Can you work these out from the model? Positions are in its coordinate system, mm. A direction names the side the tool comes from. Coordinates: 2 decimals unless noted, no trailing zeros. Loops run counter-clockwise (first coordinate to the right, second up) from the corner with the lowest first, then second, coordinate; pieces in that order, holes last. Notation, with made-up numbers: (60.25, -27.5) -> (94.25, -27.5) arc R6 ccw to (94.25, -21.5) -> close; hole circle Ø2 at (-1, -5.75). An arc over 180 degrees is marked (long way). Put each result on its own line as item: value. Start each with the question number.
Item 1: We'd pull the mould along X, two halves only. Please class faces 5 (the cylindrical face through (13.1, 7.58, 2.96)), 6 (the flat face through (0, -16.5, -32)), 7 (the flat face through (-20, 0, 3)): pulls with the +X half, pulls with the -X half, needs draft (parallel to the pull), parting line crosses it, or undercut.
Item 2: If we section it at D-D on x = 6.5: Please give me the cut outline in (y, z).
Item 3: If we section it at B-B on y = 158.5: Please give me the cut outline in (x, z).
Item 4: Will these pins go through, and if not, where does the flat tip stop? P1, Ø8, axis at x = 11.5, z = -10, coming from the +Y side; P2, Ø4.5, axis at x = -15, y = 7.5, coming from the -Z side; P3, Ø3, axis at x = 4, z = 1.5, coming from the -Y side; P4, Ø8, axis at x = -10.5, y = 13, coming from the +Z side.
Item 5: If we section it at C-C on z = -39: Please give me the cut outline in (x, y), plus the area to 3 significant figures.
Item 6: For faces 1 (the flat face through (10, 64, -32)), 2 (the flat face through (16, 153, -10)), 3 (the flat face through (-10, 65, -32)), 4 (the flat face through (0, -12.5, 3)), which set-ups out of +Z, -Z, +X, -X, +Y, -Y let a thin tool reach every point of the face, with its end or its side?
Item 7: Please list where these lines run through material, in increasing order: L1, parallel to Y at x = -15, z = 3.4; L2, parallel to X at y = -7, z = 2; L3, parallel to Y at x = 1.5, z = -49. Write a range as from..to.
Item 8: If we section it at A-A on z = -12.5: Please give me the cut outline in (x, y), plus the area to 3 significant figures.
```python
from build123d import *

# Parameters (mm, degrees)
SKETCH1_R                = 1.9
BOSS_EXTRUDE1_DEPTH      = 6
SKETCH2_W                = 18
SKETCH2_H                = 13
BOSS_EXTRUDE2_DEPTH      = 32
BOSS_EXTRUDE3_DEPTH      = 10
BOSS_EXTRUDE3_DEPTH_BACK = 150
SKETCH4_W                = 20
SKETCH4_H                = 26
BOSS_EXTRUDE4_DEPTH      = 10
BOSS_EXTRUDE4_DEPTH_BACK = 35
SKETCH5_R                = 19
SKETCH5_R_2              = 15
FILLET1_R                = 0.8


with BuildPart() as part:
    # Sketch1 → Boss-Extrude1 (new body)
    with BuildSketch(Plane.XY):
        with BuildLine():
            Line((-16, 12.5), (16, 12.5))
            ThreePointArc((16, 12.5), (18.828427125, 11.328427125), (20, 8.5))
            Line((20, 8.5), (20, -8.5))
            ThreePointArc((20, -8.5), (18.828427125, -11.328427125), (16, -12.5))
            Line((16, -12.5), (-16, -12.5))
            ThreePointArc((-16, -12.5), (-18.828427125, -11.328427125), (-20, -8.5))
            Line((-20, -8.5), (-20, 8.5))
            ThreePointArc((-20, 8.5), (-18.828427125, 11.328427125), (-16, 12.5))
        make_face()
        with Locations((-15, 7.5)):
            Circle(SKETCH1_R, mode=Mode.SUBTRACT)
        with Locations((15, 7.5)):
            Circle(SKETCH1_R, mode=Mode.SUBTRACT)
        with Locations((15, -7.5)):
            Circle(SKETCH1_R, mode=Mode.SUBTRACT)
        with Locations((-15, -7.5)):
            Circle(SKETCH1_R, mode=Mode.SUBTRACT)
    extrude(amount=BOSS_EXTRUDE1_DEPTH)

    # Sketch2 → Boss-Extrude2 (add)
    with BuildSketch(Plane(origin=(0, 0, 0), x_dir=(-1, 0, 0), z_dir=(0, 0, -1))):
        Rectangle(SKETCH2_W, SKETCH2_H)
    extrude(amount=BOSS_EXTRUDE2_DEPTH)

    # Sketch4 → Boss-Extrude3 (add, two sides: drawn at the far end of the back side and taken through both)
    with BuildSketch(Plane(origin=(0, -6.5, 0), x_dir=(-1, 0, 0), z_dir=(0, -1, 0)).offset(-BOSS_EXTRUDE3_DEPTH_BACK)):
        with Locations((0, 32)):
            Rectangle(SKETCH4_W, SKETCH4_H)
    extrude(amount=BOSS_EXTRUDE3_DEPTH + BOSS_EXTRUDE3_DEPTH_BACK)

    # Sketch5 → Boss-Extrude4 (add, two sides: drawn at the far end of the back side and taken through both)
    with BuildSketch(Plane(origin=(0, 0, -45), x_dir=(-1, 0, 0), z_dir=(0, 0, -1)).offset(-BOSS_EXTRUDE4_DEPTH_BACK)):
        with Locations((-1.66190379, 158.5)):
            Circle(SKETCH5_R)
        with Locations((-1.66190379, 158.5)):
            Circle(SKETCH5_R_2, mode=Mode.SUBTRACT)
    extrude(amount=BOSS_EXTRUDE4_DEPTH + BOSS_EXTRUDE4_DEPTH_BACK)

    # Fillet1
    fillet1_edges = [part.edges().sort_by_distance(p)[0] for p in [
        (-9, -6.5, -9.5),
        (9, -6.5, -9.5),
        (9, 6.5, -9.5),
        (-9, 6.5, -9.5),
        (-10, 63.5, -19),
        (-10, 63.5, -45),
        (10, -16.5, -32),
        (0, -16.5, -19),
        (-10, -16.5, -32),
        (0, -16.5, -45),
        (10, 62.463663672, -45),
        (10, 62.463663672, -19),
    ]]
    fillet(fillet1_edges, radius=FILLET1_R)


solid = part.part
```
Solutions:
1. face 5: undercut
1. face 6: needs draft
1. face 7: pulls with the -X half
2. outline: (-16.5, -44.2) arc R0.8 ccw to (-15.7, -45) -> (140.13, -45) -> (140.13, -55) -> (144.3, -55) -> (144.3, -10) -> (140.13, -10) -> (140.13, -19) -> (6.5, -19) -> (6.5, 0) -> (12.5, 0) -> (12.5, 6) -> (-12.5, 6) -> (-12.5, 0) -> (-6.5, 0) -> (-6.5, -19) -> (-15.7, -19) arc R0.8 ccw to (-16.5, -19.8) -> close; (172.7, -55) -> (176.87, -55) -> (176.87, -10) -> (172.7, -10) -> close
3. outline: (-17.34, -55) -> (-13.34, -55) -> (-13.34, -10) -> (-17.34, -10) -> close; (16.66, -55) -> (20.66, -55) -> (20.66, -10) -> (16.66, -10) -> close
4. P1: y = 176.58
4. P2: z = 0
4. P3: y = -12.5
4. P4: z = 6
5. outline: (-10, -15.7) arc R0.8 ccw to (-9.2, -16.5) -> (9.2, -16.5) arc R0.8 ccw to (10, -15.7) -> (10, 141.43) arc R19 ccw (long way) to (-10, 143.5) -> close; hole circle Ø30 at (1.66, 158.5)
5. area: 3,570 mm^2
6. face 1: -Z, +X, -Y
6. face 2: +Z, +X, -X, +Y
6. face 3: -Z, -X, -Y
6. face 4: +Z, +X, -X, -Y
7. L1: -12.5..-9.4, -5.6..5.6, 9.4..12.5
7. L2: -20..-16.83, -13.17..13.17, 16.83..20
7. L3: 139.5..143.5, 173.5..177.5
8. outline: circle Ø38 at (1.66, 158.5); (-9, -5.7) arc R0.8 ccw to (-8.2, -6.5) -> (8.2, -6.5) arc R0.8 ccw to (9, -5.7) -> (9, 5.7) arc R0.8 ccw to (8.2, 6.5) -> (-8.2, 6.5) arc R0.8 ccw to (-9, 5.7) -> close; hole circle Ø30 at (1.66, 158.5)
8. area: 661 mm^2
